Here's the drawing with two shaded views (mm, measured from the low corner). I have some questions. A direction names the side the tool comes from. Round coordinates to 2 decimals unless told otherwise and drop trailing zeros. Loops run counter-clockwise (first coordinate to the right, second up) from the corner with the lowest first, then second, coordinate; pieces in that order, holes last. Notation, with made-up numbers: (83.25, 63) -> (116.25, 63) arc R22 cw to (116.25, 101) -> close; hole circle Ø10 at (-32, 20.25). An arc over 180 degrees is marked (long way). Write each question's results on one line, items separated by ' | '.
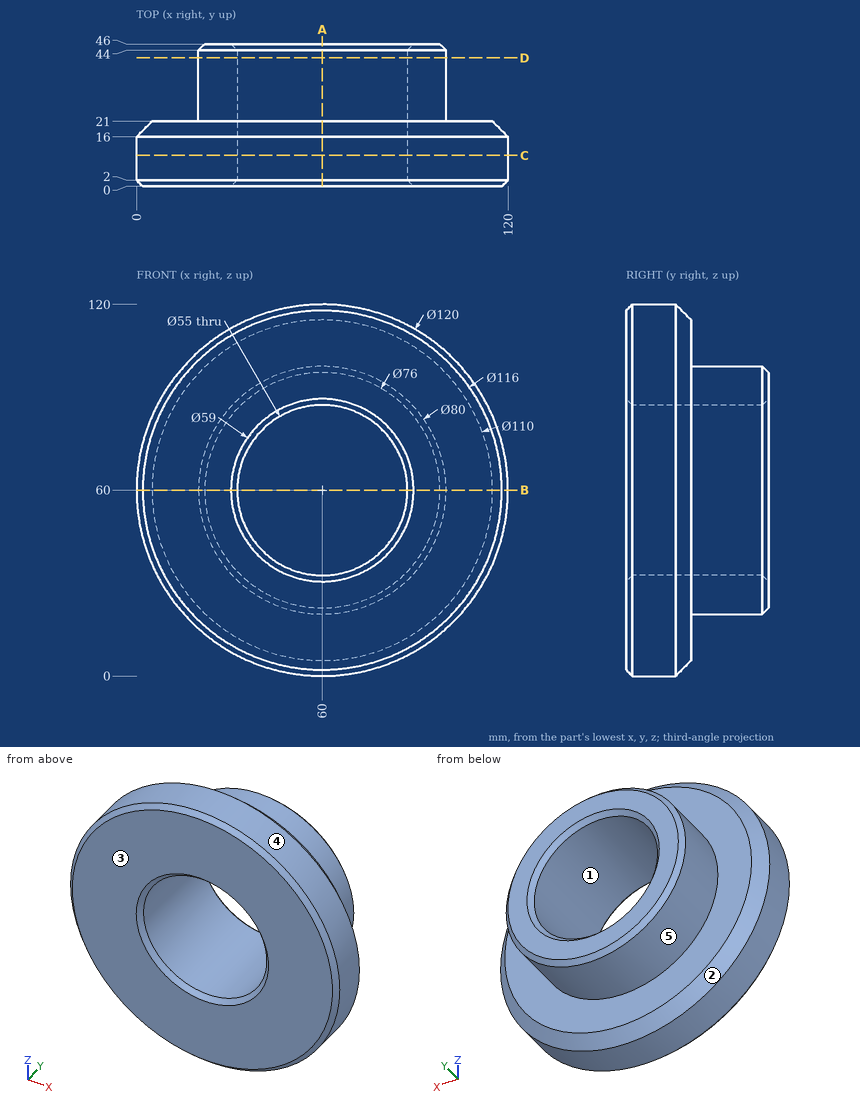
1. If we section it at D-D (y = 41.5): List the corners of the cut face in (x, z) for me.
Final values:
outline: circle Ø80 at (60, 60); hole circle Ø55 at (60, 60)
2. If we section it at B-B (z = 60): List the corners of the cut face in (x, y) for me, then the cut area to 3 significant figures.
Final values:
outline: (0, 2) -> (2, 0) -> (30.5, 0) -> (32.5, 2) -> (32.5, 44) -> (30.5, 46) -> (22, 46) -> (20, 44) -> (20, 21) -> (5, 21) -> (0, 16) -> close; (87.5, 2) -> (89.5, 0) -> (118, 0) -> (120, 2) -> (120, 16) -> (115, 21) -> (100, 21) -> (100, 44) -> (98, 46) -> (89.5, 46) -> (87.5, 44) -> close | area: 1,950 mm2
3. Will these pins go through, and if not, where does the flat tip stop? pin 1 (1 mm diameter, centred on x = 66, y = 28, fed in from +Z); pin 2 (3 mm diameter, centred on x = 97.5, y = 13.5, fed in from -Z); pin 3 (10 mm diameter, centred on y = 39, z = 95.5, fed in from +X); pin 4 (10 mm diameter, centred on x = 108, y = 39.5, fed in from +Z).
Final values:
pin 1: z = 99.62 | pin 2: z = 12 | pin 3: x = 85.88 | pin 4: through
4. If we section it at C-C (y = 10): List the corners of the cut face in (x, z) for me.
Final values:
outline: circle Ø120 at (60, 60); hole circle Ø55 at (60, 60)
5. If we section it at A-A (x = 60): List the corners of the cut face in (y, z) for me.
Final values:
outline: (0, 2) -> (2, 0) -> (16, 0) -> (21, 5) -> (21, 20) -> (44, 20) -> (46, 22) -> (46, 30.5) -> (44, 32.5) -> (2, 32.5) -> (0, 30.5) -> close; (0, 89.5) -> (2, 87.5) -> (44, 87.5) -> (46, 89.5) -> (46, 98) -> (44, 100) -> (21, 100) -> (21, 115) -> (16, 120) -> (2, 120) -> (0, 118) -> close
6. Please list where these lines run through material, in increasing order: line 1 (Z direction, x = 60, y = 12); line 2 (X direction, y = 25.5, z = 60). Write a range as from..to.
Final values:
line 1: 0..32.5, 87.5..120 | line 2: 20..32.5, 87.5..100
7. On a 3-axis mill with a long thin cutter (end or side, diameter ignored), from which of +Z, -Z, +X, -X, +Y, -Y can I reach the whole of each face in a straight line? I mean the marked faces 4 and 5. Say none if no direction works.
Final values:
face 4: +Y, -Y | face 5: +Y
8. We'd pull the mould along X, two halves only. Please class the marked faces 1, 2 and 3: pulls with the +X half, pulls with the -X half, needs draft (parallel to the pull), parting line crosses it, or undercut.
Final values:
face 1: undercut | face 2: parting line crosses it | face 3: needs draft
